```python
from build123d import *

# Parameters (mm, degrees)
BASE_PLATE_SKETCH_W   = 120
BASE_PLATE_SKETCH_H   = 68
BASE_PLATE_DEPTH      = 25
PIVOT_BOSS_SKETCH_R   = 19
PIVOT_BOSS_38_DEPTH   = 46
UPPER_BORE_SKETCH_R   = 15
UPPER_BORE_30_DEPTH   = 33
BORE_STEP_SKETCH_R    = 8
BORE_STEP_16_DEPTH    = 5
LOWER_BORE_SKETCH_R   = 15
LOWER_BORE_30_DEPTH   = 33
SIDE_LUG_DEPTH        = 5
LUG_HOLE_SKETCH_R     = 5
LUG_HOLE_10_DEPTH     = 10
U_SLOTS_2X20_DEPTH    = 20
SLOT_RELIEF_SKETCH_R  = 4
SLOT_RELIEF_CUT_DEPTH = 20
GUSSET_RIB_REACH      = 110.729
GUSSET_RIB_END_RADIUS = 19
GUSSET_RIB_SKETCH_W   = 12
GUSSET_RIB_SKETCH_H   = 46
RIB_TRIM_CUT_DEPTH    = 20


with BuildPart() as part:
    # Base Plate Sketch → Base Plate (new body)
    with BuildSketch(Plane(origin=(0, 0, 0), x_dir=(1, 0, 0), z_dir=(0, 1, 0))):
        Rectangle(BASE_PLATE_SKETCH_W, BASE_PLATE_SKETCH_H)
    extrude(amount=BASE_PLATE_DEPTH)

    # Pivot Boss Sketch → Pivot Boss Ø38 (add)
    with BuildSketch(Plane(origin=(0, 25, 0), x_dir=(1, 0, 0), z_dir=(0, 1, 0))):
        with Locations(Location((-33, 0, 0), (0, 0, 90))):
            Circle(PIVOT_BOSS_SKETCH_R)
    extrude(amount=PIVOT_BOSS_38_DEPTH)

    # Upper Bore Sketch → Upper Bore Ø30 (cut)
    with BuildSketch(Plane(origin=(0, 71, 0), x_dir=(1, 0, 0), z_dir=(0, 1, 0))):
        with Locations(Location((-33, 0, 0), (0, 0, 270))):
            Circle(UPPER_BORE_SKETCH_R)
    extrude(amount=-UPPER_BORE_30_DEPTH, mode=Mode.SUBTRACT)

    # Bore Step Sketch → Bore Step Ø16 (cut)
    with BuildSketch(Plane(origin=(0, 38, 0), x_dir=(1, 0, 0), z_dir=(0, 1, 0))):
        with Locations(Location((-33, 0, 0), (0, 0, 270))):
            Circle(BORE_STEP_SKETCH_R)
    extrude(amount=-BORE_STEP_16_DEPTH, mode=Mode.SUBTRACT)

    # Lower Bore Sketch → Lower Bore Ø30 (cut)
    with BuildSketch(Plane(origin=(0, 33, 0), x_dir=(1, 0, 0), z_dir=(0, 1, 0))):
        with Locations(Location((-33, 0, 0), (0, 0, 270))):
            Circle(LOWER_BORE_SKETCH_R)
    extrude(amount=-LOWER_BORE_30_DEPTH, mode=Mode.SUBTRACT)

    # Side Lug Sketch → Side Lug (add, symmetric)
    with BuildSketch(Plane.XY):
        with BuildLine():
            Line((-65, 68), (-50, 68))
            Line((-50, 68), (-50, 44))
            Line((-50, 44), (-65, 44))
            ThreePointArc((-65, 44), (-77, 56), (-65, 68))
        make_face()
    extrude(amount=SIDE_LUG_DEPTH, both=True)

    # Lug Hole Sketch → Lug Hole Ø10 (cut)
    with BuildSketch(Plane.XY.offset(5)):
        with Locations((-65, 56)):
            Circle(LUG_HOLE_SKETCH_R)
    extrude(amount=-LUG_HOLE_10_DEPTH, mode=Mode.SUBTRACT)

    # U-Slots Sketch → U-Slots 2x20 (cut)
    with BuildSketch(Plane(origin=(0, 25, 0), x_dir=(1, 0, 0), z_dir=(0, 1, 0))):
        with BuildLine():
            Line((42, 27), (60, 27))
            Line((60, 27), (60, 7))
            Line((60, 7), (42, 7))
            ThreePointArc((42, 7), (32, 17), (42, 27))
        make_face()
        with BuildLine():
            Line((42, -7), (60, -7))
            Line((60, -7), (60, -27))
            Line((60, -27), (42, -27))
            ThreePointArc((42, -27), (32, -17), (42, -7))
        make_face()
    extrude(amount=-U_SLOTS_2X20_DEPTH, mode=Mode.SUBTRACT)

    # Slot Relief Sketch → Slot Relief Cut (cut)
    with BuildSketch(Plane(origin=(0, 5, 0), x_dir=(1, 0, 0), z_dir=(0, 1, 0))):
        with Locations(Location((42, 17, 0), (0, 0, 270))):
            Circle(SLOT_RELIEF_SKETCH_R)
        with Locations(Location((42, -17, 0), (0, 0, 270))):
            Circle(SLOT_RELIEF_SKETCH_R)
    extrude(amount=-SLOT_RELIEF_CUT_DEPTH, mode=Mode.SUBTRACT)

    # Gusset Rib: up to this cylinder (the profile starts outside it)
    gusset_rib_end = Plane(origin=(-33, 48, 0), z_dir=(0, -1, 0)) * Cylinder(GUSSET_RIB_END_RADIUS, 260.458, mode=Mode.PRIVATE)
    # Gusset Rib Sketch → Gusset Rib (add, up to the surface)
    with BuildSketch(Plane(origin=(-2, 0, 0), x_dir=(0, 0, -1), z_dir=(1, 0, 0)), mode=Mode.PRIVATE) as gusset_rib_sk1:
        with Locations((0, 48)):
            Rectangle(GUSSET_RIB_SKETCH_W, GUSSET_RIB_SKETCH_H)
    gusset_rib_tool1 = extrude(gusset_rib_sk1.sketch, amount=-GUSSET_RIB_REACH, mode=Mode.PRIVATE) - gusset_rib_end
    add(gusset_rib_tool1.solids().sort_by_distance((-2, 48, 0))[0])

    # Rib Trim Sketch → Rib Trim Cut (cut)
    with BuildSketch(Plane.XY.offset(6)):
        Polygon((-14.972243623, 71), (-2, 25), (-2, 71), align=None)
    extrude(amount=-RIB_TRIM_CUT_DEPTH, mode=Mode.SUBTRACT)


solid = part.part
```
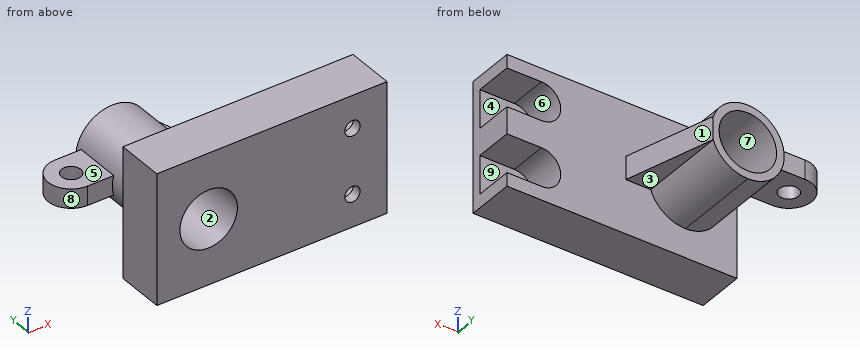
Geometry check sheet. Reference: the model listing, model coordinates, mm. Face numbers are marked on the shaded views. A direction names the side the tool comes from. Round coordinates to 2 decimals unless told otherwise and drop trailing zeros. Order: outer loops, then holes, each group sorted by start corner. A loop starts at its lowest first (then second) coordinate and runs counter-clockwise, first axis right, second up. Notation, with made-up numbers: (88, 61.5) - (110, 61.5) arc R35 cw to (110, 93.5) - close; hole circle Ø9 at (35, 54). An arc over 180 degrees is marked (long way). Use a Markdown table: item, result. Add a question column.
(1) Sectioned sample at B-B, the plane y = 18.5. Enter the section's corners in (x, z).
(2) Sectioned sample at A-A, the plane z = 0. Enter the section's corners in (x, y), and give its area (3 significant figures).
(3) Sectioned sample at D-D, the plane y = 56. Enter the section's corners in (x, z), and give its area (3 significant figures).
(4) Tool access check on the marked faces 1, 2, 3, 4 and 5. Record the directions out of +Z, -Z, +X, -X, +Y, -Y that give a thin tool (end or side, any length) a straight path to the whole face; none if there is none.
(5) Depth check by flat-ended pin: pin 1 (9 mm diameter, centred on x = -33.5, z = 6.5, fed in from +Y); pin 2 (4 mm diameter, centred on y = 22, z = 19.5, fed in from +X); pin 3 (3 mm diameter, centred on x = -56.5, z = 0, fed in from +Y); pin 4 (6.5 mm diameter, centred on x = 42, z = -17, fed in from +Y). Enter the tip coordinate at first touch or a pass-through.
(6) Sectioned sample at C-C, the plane x = 39.5. Enter the section's corners in (y, z), and give its area (3 significant figures).
(7) Material ranges on line 1 along Y through (x, z) = (32.5, 28.5); line 2 along Z through (x, y) = (-35.5, 24.5); line 3 along X through (y, z) = (34, 0), recorded low to high. Write a range as [from, to].
(8) Release check for a two-part mould opening along X. For the marked faces 6, 7, 8 and 9 record: pulls with the +X half, pulls with the -X half, needs draft (parallel to the pull), parting line crosses it, or undercut.
Answers below:
| question | item | result |
|---|---|---|
| 1 | outline | (-60, -34) - (60, -34) - (60, -27) - (42, -27) arc R10 cw to (42, -7) - (60, -7) - (60, 7) - (42, 7) arc R10 cw to (42, 27) - (60, 27) - (60, 34) - (-60, 34) - close; hole circle Ø30 at (-33, 0) |
| 2 | outline | (-65, 44) - (-52, 44) - (-52, 25) - (-60, 25) - (-60, 0) - (-48, 0) - (-48, 33) - (-41, 33) - (-41, 38) - (-48, 38) - (-48, 71) - (-52, 71) - (-52, 68) - (-65, 68) arc R12 ccw to start; (-25, 33) - (-18, 33) - (-18, 0) - (60, 0) - (60, 25) - (-2, 25) - (-14.97, 71) - (-18, 71) - (-18, 38) - (-25, 38) - close; hole circle Ø10 at (-65, 56) |
| 2 | area | 3,400 mm² |
| 3 | outline | (-77, -5) - (-70, -5) - (-70, 5) - (-77, 5) - close; (-60, -5) - (-51.33, -5) arc R19 ccw to (-14.97, -6) - (-10.74, -6) - (-10.74, 6) - (-14.97, 6) arc R19 ccw to (-51.33, 5) - (-60, 5) - close; hole circle Ø30 at (-33, 0) |
| 3 | area | 622 mm² |
| 4 | face 1 | +Z, -Z, +X, +Y |
| 4 | face 2 | -Y |
| 4 | face 3 | -Z, +X, +Y |
| 4 | face 4 | +X, +Y |
| 4 | face 5 | +Z, -X, +Y |
| 5 | pin 1 | y = 38 |
| 5 | pin 2 | x = 33.07 |
| 5 | pin 3 | y = 68 |
| 5 | pin 4 | through |
| 6 | outline | (0, -34) - (25, -34) - (25, -26.68) - (5, -26.68) - (5, -20.12) - (0, -20.12) - close; (0, -13.88) - (5, -13.88) - (5, -7.32) - (25, -7.32) - (25, 7.32) - (5, 7.32) - (5, 13.88) - (0, 13.88) - close; (0, 20.12) - (5, 20.12) - (5, 26.68) - (25, 26.68) - (25, 34) - (0, 34) - close |
| 6 | area | 863 mm² |
| 7 | line 1 | [0, 25] |
| 7 | line 2 | [-34, -14.79], [14.79, 34] |
| 7 | line 3 | [-52, -41], [-25, -4.54] |
| 8 | face 6 | pulls with the +X half |
| 8 | face 7 | undercut |
| 8 | face 8 | pulls with the -X half |
| 8 | face 9 | needs draft |
